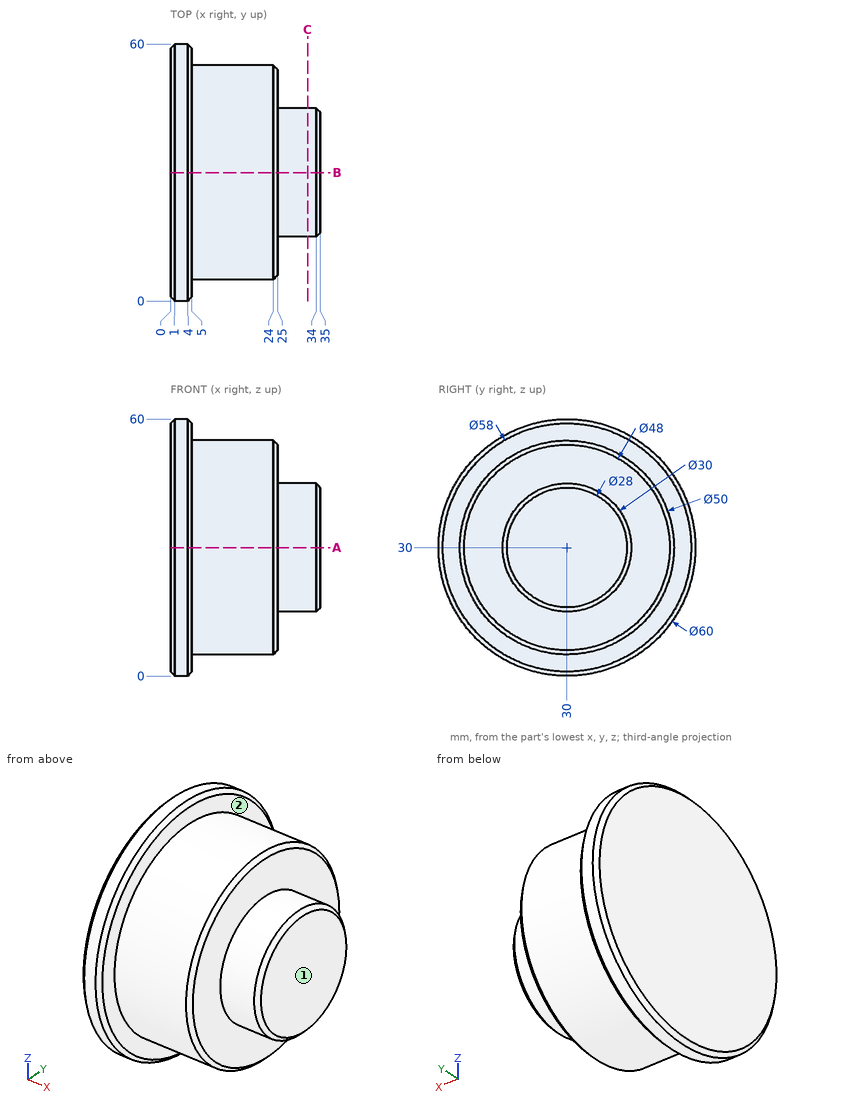
Geometry: see drawing. Coordinates: mm, zero at the bounding-box minimum. A direction names the side the tool comes from. Give positions to 0.01 mm unless a question says otherwise; leave off trailing zeros. Loops run counter-clockwise (first coordinate to the right, second up) from the corner with the lowest first, then second, coordinate; pieces in that order, holes last. Notation, with made-up numbers: (67, 5) -> (98, 5) arc R29 cw to (98, 30) -> close; hole circle Ø7 at (65.25, 82.25). An arc over 180 degrees is marked (long way). Use CSV: the item, a comma, the result in double quotes.
(1) First-contact query: P1, Ø12, axis at x = 30, z = 37.5, coming from the -Y side; P2, Ø12, axis at x = 9, y = 30.5, coming from the +Z side; P3, Ø1.5, axis at x = 21.5, y = 44.5, coming from the -Z side; P4, Ø10, axis at y = 10.5, z = 31.5, coming from the -X side. Flat tips, straight axial feed; report the tip coordinate or a pass-through.
From the geometry:
P1,"y = 5.93"
P2,"z = 60"
P3,"z = 9.12"
P4,"x = 0"
(2) Access query for the marked faces 1 and 2. Directions: +Z, -Z, +X, -X, +Y, -Y. A direction counts if a zero-diameter tool reaches every point of the face in a straight line with its end or side. Return the directions, or none.
From the geometry:
face 1,"+Z, -Z, +X, +Y, -Y"
face 2,"+X"
(3) Cut plane A-A (z = 30). Output: boundary loops of the cut face in (x, y).
From the geometry:
outline,"(0, 1) -> (1, 0) -> (4, 0) -> (5, 1) -> (5, 5) -> (24, 5) -> (25, 6) -> (25, 15) -> (34, 15) -> (35, 16) -> (35, 44) -> (34, 45) -> (25, 45) -> (25, 54) -> (24, 55) -> (5, 55) -> (5, 59) -> (4, 60) -> (1, 60) -> (0, 59) -> close"
(4) Ray query, line 1 along X through (y, z) = (50.5, 36); line 2 along Z through (x, y) = (4, 30); line 3 along Y through (x, z) = (19, 30.5) (3 decimals). Return the intervals inside material, ascending. Write a range as [from, to].
From the geometry:
line 1,"[0, 25]"
line 2,"[0, 60]"
line 3,"[5.005, 54.995]"
(5) Cut plane C-C (x = 32). Output: boundary loops of the cut face in (y, z).
From the geometry:
outline,"circle Ø30 at (30, 30)"
